```python
from build123d import *

# Parameters (mm, degrees)
CHAMFER1_SIZE      = 2
CUT_EXTRUDE2_DEPTH = 43
CHAMFER2_SIZE      = 1


with BuildPart() as part:
    # Sketch1 → Revolve1 (revolve)
    with BuildSketch(Plane.XY, mode=Mode.PRIVATE) as revolve1_sk:
        Polygon((-19, 19.05), (-19, 43), (0, 43), (0, 11), (-14.35, 11), align=None)
    revolve(revolve1_sk.sketch.rotate(Axis((-44.950542037, 0, 0), (1, 0, 0)), 90), axis=Axis((-44.950542037, 0, 0), (1, 0, 0)))

    # Chamfer1
    chamfer1_edges = [part.edges().sort_by_distance(p)[0] for p in [
        (-19, 0, -43),
        (0, 0, -43),
    ]]
    chamfer(chamfer1_edges, length=CHAMFER1_SIZE)

    # Sketch13 → Cut-Extrude2 (cut)
    with BuildSketch(Plane.ZY.offset(19)):
        Polygon((-9.5, 0), (-9.5, -65.513992054), (9.5, -73.697131866), (9.5, 0), align=None)
    extrude(amount=-CUT_EXTRUDE2_DEPTH, mode=Mode.SUBTRACT)

    # Chamfer2
    chamfer2_edges = [part.edges().sort_by_distance(p)[0] for p in [
        (-19, -28.198199933, -9.5),
        (-19, -28.198199933, 9.5),
        (0, -22.714737827, -9.5),
        (0, 11, 0),
        (0, -22.714737827, 9.5),
    ]]
    chamfer(chamfer2_edges, length=CHAMFER2_SIZE)


solid = part.part
```
Read the model definition and answer for the solid it produces. Units are mm, in the model's axes. A direction names the side the tool comes from. Coordinates: 2 decimals unless noted, no trailing zeros. Write each loop counter-clockwise with the first axis right and the second up, starting at its lowest first coordinate (ties: lowest second). Pieces come first, ordered by that corner, then holes. Notation, with made-up numbers: (65, 36) - (90, 36) arc R24 ccw to (90, 69) - close; hole circle Ø7 at (24.5, 33). An arc over 180 degrees is marked (long way). Answer as a JSON object with one key per item and string values. Group by question number.
1. Each of these flat-tipped pins is pushed along its axis until it touches: P1, Ø8, axis at x = -13, z = 26.5, coming from the +Y side; P2, Ø4, axis at x = -12, y = 26.5, coming from the -Z side; P3, Ø5, axis at x = -6, y = -30.5, coming from the -Z side. Where does it stop, or does it pass through?
2. A cutting plane is placed at A-A (y = 0). Determine the outline of the cut face in (x, z), plus the area to 3 significant figures.
3. The mould has two halves that part along Z. Classify faces 3 (the conical face through (-0.319, 41.285, -1.688)), 4 (the flat face through (-10, -24, 9.5)), 5 (the flat face through (-19, 18, -9)): +Z half, -Z half, draft (parallel to the pull), parting line (faces both ways), or undercut.
4. Which of the six approach directions +Z, -Z, +X, -X, +Y, -Y give full straight-line access (tool end or side, diameter ignored) to faces 1 (the conical face through (-0.84, 11.155, -0.328)), 2 (the flat face through (-10, -23, -9.5))?
5. A cutting plane is placed at B-B (z = 0). Determine the outline of the cut face in (x, y).
6. A cutting plane is placed at C-C (x = -7). Determine the outline of the cut face in (y, z), plus the area to 3 significant figures.
7. Consider L1, parallel to Z at x = -6.75, y = 0; L2, parallel to Y at x = -10.5, z = 0; L3, parallel to Z at x = -14.75, y = -10.5. Determine where each line is inside the solid, lowest interval first. Write a range as [from, to].
Worked out:
{
 "1": {"P1": "stops at y = 36.64", "P2": "stops at z = -35.34", "P3": "stops at z = -32.63"},
 "2": {"outline": "(-19, -41) - (-17, -43) - (-2, -43) - (0, -41) - (0, -12) - (-1, -11) - (-14.35, -11) - (-19, -19.05) - close; (-19, 19.05) - (-14.35, 11) - (-1, 11) - (0, 12) - (0, 41) - (-2, 43) - (-17, 43) - (-19, 41) - close", "area": "1,170 mm²"},
 "3": {"face 3": "parting line", "face 4": "undercut", "face 5": "draft"},
 "4": {"face 1": "+X", "face 2": "+X, -X, -Y"},
 "5": {"outline": "(-19, 19.05) - (-14.35, 11) - (-1, 11) - (0, 12) - (0, 41) - (-2, 43) - (-17, 43) - (-19, 41) - close"},
 "6": {"outline": "(-41.94, -9.5) arc R43 ccw (long way) to (-41.94, 9.5) - (-5.55, 9.5) arc R11 cw (long way) to (-5.55, -9.5) - close", "area": "4,800 mm²"},
 "7": {"L1": "z = [-43, -11], [11, 43]", "L2": "y = [11, 43]", "L3": "z = [-41.7, -9.5], [9.5, 41.7]"}
}
